from build123d import *

# Parameters (mm, degrees)
CUT_EXTRUDE_1_REACH = 22.273
SKETCH_4_R          = 3
SKETCH_6_R          = 5
SKETCH_6_R_2        = 3


with BuildPart() as part:
    # 草图1 → 旋转1 (revolve)
    with BuildSketch(Plane.XY, mode=Mode.PRIVATE) as revolve_1_sk:
        Polygon((-5, 4), (-4.5, 7), (-5, 7), (-5, 8), (-4.5, 11), (-5, 11), (-5, 12), (-4.5, 15), (-5, 15), (-5, 16), (-4.5, 19), (0, 19), (0, 0), (-5, 0), align=None)
    revolve(revolve_1_sk.sketch.rotate(Axis((0, 0, 0), (0, 1, 0)), 270), axis=Axis((0, 0, 0), (0, 1, 0)))

    # 草图4 → 切除-拉伸1 (cut, up to next)
    with BuildSketch(Plane(origin=(0, 19, 0), x_dir=(1, 0, 0), z_dir=(0, 1, 0)), mode=Mode.PRIVATE) as cut_extrude_1_sk1:
        with Locations(Location((0, 0, 0), (0, 0, 180))):
            Circle(SKETCH_4_R)
    cut_extrude_1_tool1 = extrude(cut_extrude_1_sk1.sketch, amount=-CUT_EXTRUDE_1_REACH, mode=Mode.PRIVATE) & part.part
    add(cut_extrude_1_tool1.solids().sort_by_distance((0, 19, 0))[0], mode=Mode.SUBTRACT)

    # 扫描1: sweep along a path in 草图5
    with BuildLine(Plane.XY) as sweep_1_path:
        Line((21, -7), (7, -7))
        ThreePointArc((7, -7), (2.050252532, -4.949747468), (0, 0))
    # 草图6 → 扫描1 (sweep)
    with BuildSketch(Plane.XZ):
        Circle(SKETCH_6_R)
        Circle(SKETCH_6_R_2, mode=Mode.SUBTRACT)
    sweep(path=sweep_1_path.line)


solid = part.part
The listing builds one solid part. Answer for the finished solid, in the listing's coordinates (mm). A direction names the side the tool comes from. Round coordinates to 2 decimals unless told otherwise and drop trailing zeros. Write each loop counter-clockwise with the first axis right and the second up, starting at its lowest first coordinate (ties: lowest second). Pieces come first, ordered by that corner, then holes. Notation, with made-up numbers: M -37.5,-33.5 L -2.5,-33.5 A20 cw -2.5,-1.5 Z; hole C -36.5,-21 d7. An arc over 180 degrees is marked long. Write each question's results on one line, items separated by ' | '. Start each with the question number.
Item 1: Find section A-A on x = 15.75. Write down the section's boundary in (y, z), and give its area (3 significant figures).
Item 2: Straight lines are drawn through the part: probe 1 along Z at (x, y) = (12.5, -7); probe 2 along X at (y, z) = (18.5, -2.5); probe 3 along Y at (x, z) = (15.25, -1.5). For each, find the intervals that lie inside material, in ascending order.
Item 3: Given pin 1 Ø2 at (y, z) = (6.5, 1) entering from -X; pin 2 Ø6 at (x, z) = (17.5, 2) entering from +Y; pin 3 Ø5 at (x, y) = (17.5, -4) entering from -Z, each flat-ended and moving along its own axis, determine where each tip first touches the part or whether it passes through.
Item 4: Find section B-B on y = 9.5. Write down the section's boundary in (x, z), and give its area (3 significant figures).
Item 5: The mould has two halves that part along Z. Classify faces 5 (the flat face through (3, 19, -1)), 6 (the cylindrical face through (4.88, 7.51, 1.08)), 7 (the cylindrical face through (13.9, -4.14, -0.9)): +Z half, -Z half, draft (parallel to the pull), parting line (faces both ways), or undercut.
Item 6: Which of the six approach directions +Z, -Z, +X, -X, +Y, -Y give full straight-line access (tool end or side, diameter ignored) to faces 1 (the cylindrical face through (4.88, 15.51, 1.08)), 2 (the cylindrical face through (13.9, -2.23, -1.5)), 3 (the flat face through (21, -7.1, 3.3)), 4 (the conical face through (-1.39, 6.19, -4.42))?
Answer block:
1) outline: C -7,0 d10; hole C -7,0 d6 | area: 50.3 mm²
2) probe 1: z = -5 to -3, 3 to 5 | probe 2: x = -3.84 to -1.66, 1.66 to 3.84 | probe 3: y = -11.77 to -9.6, -4.4 to -2.23
3) pin 1: stops at x = -5 | pin 2: stops at y = -2 | pin 3: stops at z = -4.97
4) outline: C 0,0 d9.5; hole C 0,0 d6 | area: 42.6 mm²
5) face 5: draft | face 6: parting line | face 7: undercut
6) face 1: +Y | face 2: +X | face 3: +Z, -Z, +X, +Y, -Y | face 4: none
